For this review, take the finished solid that the model builds, in its own axes (mm). Face numbers are marked on the shaded views. A direction names the side the tool comes from. Round coordinates to 2 decimals unless told otherwise and drop trailing zeros. Loops run counter-clockwise (first coordinate to the right, second up) from the corner with the lowest first, then second, coordinate; pieces in that order, holes last.
1. Draft analysis for pull direction Z (two halves, no side actions). For the marked faces 4, 5 and 6, state which applies: released by +Z, released by -Z, zero draft, split by the parting line, or undercut.
2. Consider section A-A on x = 36.5. State the section outline as (y, z) points.
3. Tool access review of the marked faces 1, 2 and 3: name each direction out of +Z, -Z, +X, -X, +Y, -Y from which nothing blocks a thin tool from reaching the whole face with its end or side.
4. Clearance check with flat-ended pins moving along their axes: pin 1 Ø4.5 at (y, z) = (-1, 0.5) entering from +X; pin 2 Ø4 at (y, z) = (0, 0) entering from -X; pin 3 Ø5 at (x, y) = (17, -5.5) entering from -Z; pin 4 Ø8 at (x, y) = (45, -10) entering from +Z. State where each tip first meets the part, or that it passes through.
5. To check wall thickness, follow line 1 along Y through (x, z) = (1.6, 0); line 2 along Y through (x, z) = (3.65, 0); line 3 along X through (y, z) = (10.75, 3). State the ranges of each line that lie inside material, in increasing order.
from build123d import *

# Parameters (mm, degrees)
SKETCH1_R             = 8
BOSS_EXTRUDE1_DEPTH   = 11
SKETCH2_R             = 12.5
BOSS_EXTRUDE2_DEPTH   = 15
SKETCH3_R             = 5.5
BOSS_EXTRUDE3_DEPTH   = 46
SKETCH5_R             = 5.5
CUT_EXTRUDE1_DEPTH    = 11
CUT_EXTRUDE2_START    = -2.7
SKETCH6_R             = 6
CUT_EXTRUDE2_DEPTH    = 1.1
SKETCH7_R             = 5
CUT_EXTRUDE3_DEPTH    = 10.2
SKETCH8_R             = 3
CUT_EXTRUDE4_DEPTH    = 15
M8_TAPPED_HOLE1_D     = 6.8
M8_TAPPED_HOLE1_DEPTH = 11
M8_TAPPED_HOLE1_TIP   = 2.042926105
BOSS_EXTRUDE4_START   = -16
SKETCH11_R            = 5.5
BOSS_EXTRUDE4_DEPTH   = 5
SKETCH12_R            = 2.75
CUT_EXTRUDE5_DEPTH    = 5
SKETCH13_R            = 1.5
CUT_EXTRUDE6_DEPTH    = 88
CHAMFER1_SIZE         = 0.5


with BuildPart() as part:
    # Sketch1 → Boss-Extrude1 (new body)
    with BuildSketch(Plane(origin=(0, 0, 0), x_dir=(0, 0, -1), z_dir=(1, 0, 0))):
        Circle(SKETCH1_R)
    extrude(amount=BOSS_EXTRUDE1_DEPTH)

    # Sketch2 → Boss-Extrude2 (add)
    with BuildSketch(Plane(origin=(11, 0, 0), x_dir=(0, 0, -1), z_dir=(1, 0, 0))):
        Circle(SKETCH2_R)
    extrude(amount=BOSS_EXTRUDE2_DEPTH)

    # Sketch3 → Boss-Extrude3 (add)
    with BuildSketch(Plane(origin=(26, 0, 0), x_dir=(0, 0, -1), z_dir=(1, 0, 0))):
        Circle(SKETCH3_R)
    extrude(amount=BOSS_EXTRUDE3_DEPTH)

    # Sketch5 → Cut-Extrude1 (cut)
    with BuildSketch(Plane.ZY):
        with Locations(Location((0, 0, 0), (0, 0, 180))):
            Circle(SKETCH5_R)
    extrude(amount=-CUT_EXTRUDE1_DEPTH, mode=Mode.SUBTRACT)

    # Sketch6 → Cut-Extrude2 (cut)
    with BuildSketch(Plane.ZY.offset(CUT_EXTRUDE2_START)):
        Circle(SKETCH6_R)
    extrude(amount=-CUT_EXTRUDE2_DEPTH, mode=Mode.SUBTRACT)

    # Sketch7 → Cut-Extrude3 (cut)
    with BuildSketch(Plane.ZY.offset(-3.8)):
        Circle(SKETCH7_R)
    extrude(amount=-CUT_EXTRUDE3_DEPTH, mode=Mode.SUBTRACT)

    # Sketch8 → Cut-Extrude4 (cut)
    with BuildSketch(Plane.ZY.offset(-14)):
        Circle(SKETCH8_R)
    extrude(amount=-CUT_EXTRUDE4_DEPTH, mode=Mode.SUBTRACT)

    # M8 Tapped Hole1
    with Locations(Plane(origin=(72, 0, 0), x_dir=(0, 0, -1), z_dir=(1, 0, 0))):
        with Locations((0, 0)):
            Hole(M8_TAPPED_HOLE1_D / 2, depth=M8_TAPPED_HOLE1_DEPTH)
            with Locations((0, 0, -(M8_TAPPED_HOLE1_DEPTH + M8_TAPPED_HOLE1_TIP / 2))):  # 118° drill point
                Cone(0, M8_TAPPED_HOLE1_D / 2, M8_TAPPED_HOLE1_TIP, mode=Mode.SUBTRACT)

    # Sketch11 → Boss-Extrude4 (add)
    with BuildSketch(Plane(origin=(72, 0, 0), x_dir=(0, 0, -1), z_dir=(1, 0, 0)).offset(BOSS_EXTRUDE4_START)):
        Circle(SKETCH11_R)
    extrude(amount=BOSS_EXTRUDE4_DEPTH)

    # Sketch12 → Cut-Extrude5 (cut)
    with BuildSketch(Plane(origin=(61, 0, 0), x_dir=(0, 0, -1), z_dir=(1, 0, 0))):
        Circle(SKETCH12_R)
    extrude(amount=-CUT_EXTRUDE5_DEPTH, mode=Mode.SUBTRACT)

    # Sketch13 → Cut-Extrude6 (cut)
    with BuildSketch(Plane(origin=(56, 0, 0), x_dir=(0, 0, -1), z_dir=(1, 0, 0))):
        Circle(SKETCH13_R)
    extrude(amount=-CUT_EXTRUDE6_DEPTH, mode=Mode.SUBTRACT)

    # Chamfer1
    chamfer1_edges = [part.edges().sort_by_distance(p)[0] for p in [
        (72, 0, 5.5),
        (0, 0, 8),
        (11, 0, 12.5),
        (26, 0, 12.5),
    ]]
    chamfer(chamfer1_edges, length=CHAMFER1_SIZE)


solid = part.part
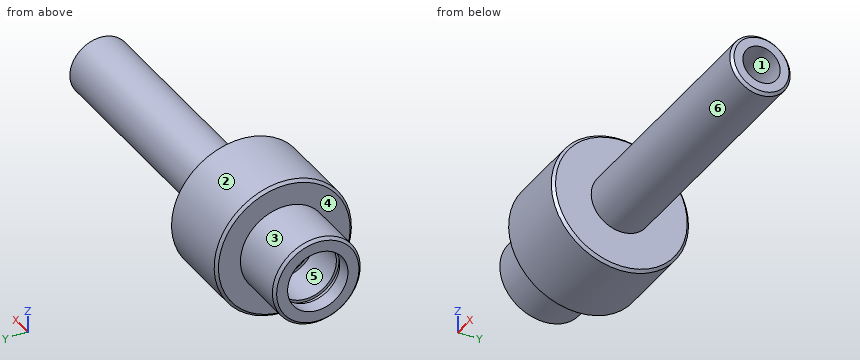
Resolved:
1. face 4: zero draft
1. face 5: undercut
1. face 6: split by the parting line
2. outline: circle Ø11 at (0, 0); hole circle Ø3 at (0, 0)
3. face 1: +X
3. face 2: +X, -X
3. face 3: -X
4. pin 1: stops at x = 61
4. pin 2: stops at x = 29
4. pin 3: stops at z = -12.13
4. pin 4: passes through
5. line 1: y = -8 to -5.5, 5.5 to 8
5. line 2: y = -8 to -6, 6 to 8
5. line 3: x = 11 to 26
